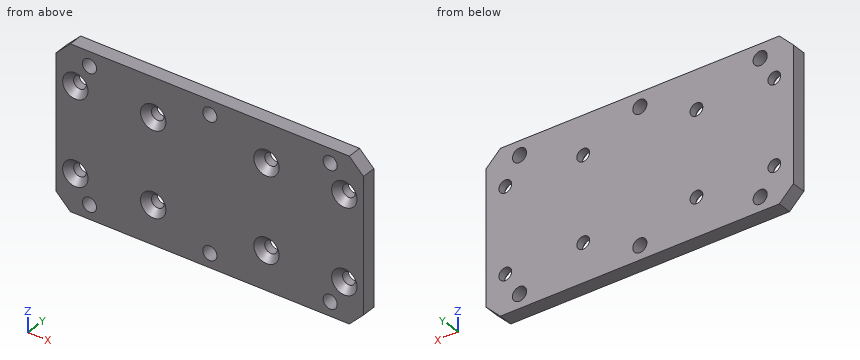
from build123d import *

# Parameters (mm, degrees)
SKETCH_1_W                   = 217
SKETCH_1_H                   = 115
EXTRUDE_1_DEPTH              = 10
HOLE_WIZARD_M8_1_D           = 9
HOLE_WIZARD_M8_1_CSINK_D     = 17.92
HOLE_WIZARD_M8_1_CSINK_ANGLE = 90
HOLE_WIZARD_M8_2_D           = 10
CHAMFER_1_SIZE               = 10


with BuildPart() as part:
    # 草图1 → 凸台-拉伸1 (new body)
    with BuildSketch(Plane(origin=(0, 0, 0), x_dir=(1, 0, 0), z_dir=(0, 1, 0))):
        Rectangle(SKETCH_1_W, SKETCH_1_H)
    extrude(amount=EXTRUDE_1_DEPTH)

    # M8 六角凹锥坑螺钉的锥形沉头孔1 (through all)
    with Locations(Plane(origin=(0, 0, 0), x_dir=(-1, 0, 0), z_dir=(0, -1, 0))):
        with Locations((-95, -30), (-40, -30), (40, -30), (95, -30), (95, 30), (40, 30), (-40, 30), (-95, 30)):
            CounterSinkHole(HOLE_WIZARD_M8_1_D / 2, HOLE_WIZARD_M8_1_CSINK_D / 2, counter_sink_angle=HOLE_WIZARD_M8_1_CSINK_ANGLE)

    # M8 间隙孔2 (through all)
    with Locations(Plane(origin=(0, 0, 0), x_dir=(-1, 0, 0), z_dir=(0, -1, 0))):
        with Locations((-85, 47.5), (0, 47.5), (85, 47.5), (85, -47.5), (0, -47.5), (-85, -47.5)):
            Hole(HOLE_WIZARD_M8_2_D / 2)

    # 倒角1
    chamfer_1_edges = [part.edges().sort_by_distance(p)[0] for p in [
        (108.5, 5, 57.5),
        (-108.5, 5, 57.5),
        (-108.5, 5, -57.5),
        (108.5, 5, -57.5),
    ]]
    chamfer(chamfer_1_edges, length=CHAMFER_1_SIZE)


solid = part.part
Can you work these out from the model? Positions are in its coordinate system, mm. Round coordinates to 2 decimals unless told otherwise and drop trailing zeros. Write each loop counter-clockwise with the first axis right and the second up, starting at its lowest first coordinate (ties: lowest second). Pieces come first, ordered by that corner, then holes. Notation, with made-up numbers: (58, 19) -> (106, 19) arc R18 cw to (106, 35) -> close; hole circle Ø4 at (66.5, 18). An arc over 180 degrees is marked (long way). One line per question, with ' | ' between items. Start each with the question number.
1) Suppose I cut it at D-D on z = 45. Write out the boundary of the cut face in (x, y).
2) Suppose I cut it at C-C on x = -40. Write out the boundary of the cut face in (y, z).
3) Suppose I cut it at B-B on y = 7.5. Count the separate pieces of the cut face and the enclosed holes in it, then the cut area to 3 significant figures.
4) I'm going to push flat-ended pins straight in: P1, Ø10.5, axis at x = -95, z = 30, coming from the -Y side; P2, Ø8, axis at x = -40, z = -30, coming from the +Y side (3 decimals); P3, Ø11.5, axis at x = -95, z = -30, coming from the -Y side. Where does each tip first touch, or does it pass through?
5) Suppose I cut it at A-A on z = 30. Write out the boundary of the cut face in (x, y).
6) I need wall thicknesses on line 1 (Z direction, x = -95, y = 6.2); line 2 (X direction, y = 3, z = 47.5); line 3 (X direction, y = 6.2, z = -30). Which ranges of each line are inside material? Lowest first, please. Write a range as [from, to].
Return value:
1) outline: (-108.5, 0) -> (-89.33, 0) -> (-89.33, 10) -> (-108.5, 10) -> close; (-80.67, 0) -> (-4.33, 0) -> (-4.33, 10) -> (-80.67, 10) -> close; (4.33, 0) -> (80.67, 0) -> (80.67, 10) -> (4.33, 10) -> close; (89.33, 0) -> (108.5, 0) -> (108.5, 10) -> (89.33, 10) -> close
2) outline: (0, -57.5) -> (10, -57.5) -> (10, -34.5) -> (4.46, -34.5) -> (0, -38.96) -> close; (0, -21.04) -> (4.46, -25.5) -> (10, -25.5) -> (10, 25.5) -> (4.46, 25.5) -> (0, 21.04) -> close; (0, 38.96) -> (4.46, 34.5) -> (10, 34.5) -> (10, 57.5) -> (0, 57.5) -> close
3) separate pieces: 1 | enclosed holes: 14 | area: 23,800 mm2
4) P1: stops at y = 3.71 | P2: passes through | P3: stops at y = 3.21
5) outline: (-108.5, 0) -> (-103.96, 0) -> (-99.5, 4.46) -> (-99.5, 10) -> (-108.5, 10) -> close; (-90.5, 4.46) -> (-86.04, 0) -> (-48.96, 0) -> (-44.5, 4.46) -> (-44.5, 10) -> (-90.5, 10) -> close; (-35.5, 4.46) -> (-31.04, 0) -> (31.04, 0) -> (35.5, 4.46) -> (35.5, 10) -> (-35.5, 10) -> close; (44.5, 4.46) -> (48.96, 0) -> (86.04, 0) -> (90.5, 4.46) -> (90.5, 10) -> (44.5, 10) -> close; (99.5, 4.46) -> (103.96, 0) -> (108.5, 0) -> (108.5, 10) -> (99.5, 10) -> close
6) line 1: z = [-57.5, -34.5], [-25.5, 25.5], [34.5, 57.5] | line 2: x = [-108.5, -90], [-80, -5], [5, 80], [90, 108.5] | line 3: x = [-108.5, -99.5], [-90.5, -44.5], [-35.5, 35.5], [44.5, 90.5], [99.5, 108.5]
